Read the model definition and answer for the solid it produces. Units are mm, in the model's axes. A direction names the side the tool comes from. Round coordinates to 2 decimals unless told otherwise and drop trailing zeros. Loops run counter-clockwise (first coordinate to the right, second up) from the corner with the lowest first, then second, coordinate; pieces in that order, holes last. Notation, with made-up numbers: M 64,71 L 93,71 A11 cw 93,89 Z; hole C 55,28 d4. An arc over 180 degrees is marked long. Write each question's results on one line, items separated by ' | '.
from build123d import *

# Parameters (mm, degrees)
SKETCH1_W                  = 50
SKETCH1_H                  = 10
BOSS_EXTRUDE1_DEPTH        = 2
F_3_5_3_5_DIAMETER_HOLE1_D = 3.5
CHAMFER1_SIZE              = 1
CUT_EXTRUDE1_DEPTH         = 2


with BuildPart() as part:
    # Sketch1 → Boss-Extrude1 (new, symmetric)
    with BuildSketch(Plane(origin=(0, 0, 0), x_dir=(1, 0, 0), z_dir=(0, 1, 0))):
        Rectangle(SKETCH1_W, SKETCH1_H)
    extrude(amount=BOSS_EXTRUDE1_DEPTH, both=True)

    # Ø3.5 (3.5) Diameter Hole1 (through all)
    with Locations(Plane(origin=(0, 2, 0), x_dir=(1, 0, 0), z_dir=(0, 1, 0))):
        with Locations((-22, 0), (22, 0)):
            Hole(F_3_5_3_5_DIAMETER_HOLE1_D / 2)

    # Chamfer1
    chamfer1_edges = [part.edges().sort_by_distance(p)[0] for p in [
        (25, 0, 5),
        (-25, 0, 5),
        (-25, 0, -5),
        (25, 0, -5),
    ]]
    chamfer(chamfer1_edges, length=CHAMFER1_SIZE)

    # Sketch4 → Cut-Extrude1 (cut)
    with BuildSketch(Plane.XZ.offset(2)):
        with BuildLine():
            Line((-17, 3.5), (17, 3.5))
            ThreePointArc((17, 3.5), (18.414213562, 2.914213562), (19, 1.5))
            Line((19, 1.5), (19, -1.5))
            ThreePointArc((19, -1.5), (18.414213562, -2.914213562), (17, -3.5))
            Line((17, -3.5), (-17, -3.5))
            ThreePointArc((-17, -3.5), (-18.414213562, -2.914213562), (-19, -1.5))
            Line((-19, -1.5), (-19, 1.5))
            ThreePointArc((-19, 1.5), (-18.414213562, 2.914213562), (-17, 3.5))
        make_face()
    extrude(amount=-CUT_EXTRUDE1_DEPTH, mode=Mode.SUBTRACT)


solid = part.part
Item 1: The part is cut by section A-A (x = -22). Determine the outline of the cut face in (y, z), plus the area to 3 significant figures.
Outcome:
outline: M -2,-5 L 2,-5 L 2,-1.75 L -2,-1.75 Z; M -2,1.75 L 2,1.75 L 2,5 L -2,5 Z | area: 26.0 mm2
Item 2: The part is cut by section D-D (x = 10). Determine the outline of the cut face in (y, z).
Outcome:
outline: M -2,-5 L 2,-5 L 2,5 L -2,5 L -2,3.5 L 0,3.5 L 0,-3.5 L -2,-3.5 Z
Item 3: The mould has two halves that part along Z. Classify faces 1 (the face through (0, -1, -3.5)), 2 (the face through (0, 0, -5)), 3 (the face through (-24.5, 0, 4.5)), 4 (the face through (-25, 0, 0)): pulls with the +Z half, pulls with the -Z half, needs draft (parallel to the pull), parting line crosses it, or undercut.
Outcome:
face 1: undercut | face 2: pulls with the -Z half | face 3: pulls with the +Z half | face 4: needs draft
Item 4: The part is cut by section C-C (y = 0.5). Determine the outline of the cut face in (x, z).
Outcome:
outline: M -25,-4 L -24,-5 L 24,-5 L 25,-4 L 25,4 L 24,5 L -24,5 L -25,4 Z; hole C -22,0 d3.5; hole C 22,0 d3.5
Item 5: Flat-ended cylindrical pins translate along their axes: pin 1 (2 mm diameter, centred on x = -22, z = 0, fed in from +Y); pin 2 (4 mm diameter, centred on x = -5.5, z = 0.5, fed in from -Y). Find the tip coordinate at first contact, or state that the pin passes through.
Outcome:
pin 1: passes through | pin 2: stops at y = 0
Item 6: The part is cut by section B-B (z = 0). Determine the outline of the cut face in (x, y), plus the area to 3 significant figures.
Outcome:
outline: M -25,-2 L -23.75,-2 L -23.75,2 L -25,2 Z; M -20.25,-2 L -19,-2 L -19,0 L 19,0 L 19,-2 L 20.25,-2 L 20.25,2 L -20.25,2 Z; M 23.75,-2 L 25,-2 L 25,2 L 23.75,2 Z | area: 96.0 mm2
Item 7: Straight lines are drawn through the part: line 1 (Z direction, x = 22, y = -0.45); line 2 (Z direction, x = 7, y = -1.5); line 3 (X direction, y = -0.9, z = -0.5). For each, find the intervals that lie inside material, in ascending order.
Outcome:
line 1: z = -5 to -1.75, 1.75 to 5 | line 2: z = -5 to -3.5, 3.5 to 5 | line 3: x = -25 to -23.68, -20.32 to -19, 19 to 20.32, 23.68 to 25
Item 8: For faces 5 (the face through (0, -1, 3.5)), 6 (the face through (24.5, 0, -4.5)), determine the directions among +Z, -Z, +X, -X, +Y, -Y from which every point of the face is accessible in a straight line to the end or side of a thin tool.
Outcome:
face 5: -Y | face 6: -Z, +X, +Y, -Y
